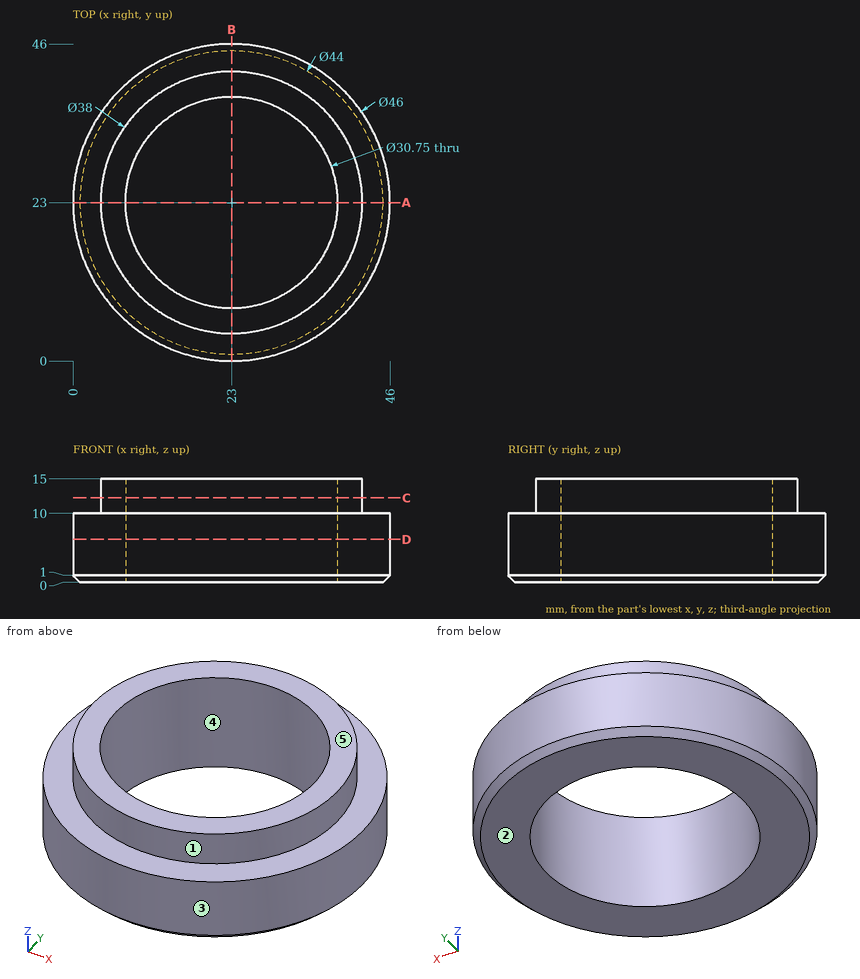
Design review of the part shown in the three views and the two pictorial views. Dimensions are in mm from the part's minimum x, y and z. A direction names the side the tool comes from. Round coordinates to 2 decimals unless told otherwise and drop trailing zeros. Loops run counter-clockwise (first coordinate to the right, second up) from the corner with the lowest first, then second, coordinate; pieces in that order, holes last.
1) Clearance check with flat-ended pins moving along their axes: P1, Ø1.5, axis at y = 34, z = 2.5, coming from the +X side; P2, Ø8, axis at y = 14, z = 11.5, coming from the +X side; P3, Ø4, axis at x = 19.5, z = 2, coming from the -Y side. State where each tip first meets the part, or that it passes through.
Values follow:
P1: stops at x = 43.59
P2: stops at x = 45.38
P3: stops at y = 0.05
2) Consider section C-C on z = 12.25. State the section outline as (x, y) points (3 decimals).
Values follow:
outline: circle Ø38 at (23, 23); hole circle Ø30.75 at (23, 23)
3) Consider section D-D on z = 6.25. State the section outline as (x, y) points (3 decimals), then the cut area to 3 significant figures.
Values follow:
outline: circle Ø46 at (23, 23); hole circle Ø30.75 at (23, 23)
area: 919 mm2
4) Consider section A-A on y = 23. State the section outline as (x, z) points (3 decimals).
Values follow:
outline: (0, 1) - (1, 0) - (7.625, 0) - (7.625, 15) - (4, 15) - (4, 10) - (0, 10) - close; (38.375, 0) - (45, 0) - (46, 1) - (46, 10) - (42, 10) - (42, 15) - (38.375, 15) - close
5) Tool access review of the marked faces 1 and 2: name each direction out of +Z, -Z, +X, -X, +Y, -Y from which nothing blocks a thin tool from reaching the whole face with its end or side.
Values follow:
face 1: +Z
face 2: -Z, +X, -X, +Y, -Y
6) Wall thickness on line 1 along Y through (x, z) = (23, 6.5) (3 decimals); line 2 along Y through (x, z) = (23, 10.75) (3 decimals); line 3 along X through (y, z) = (34.5, 14): over which ranges is each line inside the solid? List them lowest first.
Values follow:
line 1: y = 0 to 7.625, 38.375 to 46
line 2: y = 4 to 7.625, 38.375 to 42
line 3: x = 7.88 to 12.8, 33.2 to 38.12
7) The part is to be moulded in two halves that separate along Y. For the marked faces 3, 4 and 5, say which applies: pulls with the +Y half, pulls with the -Y half, needs draft (parallel to the pull), parting line crosses it, or undercut.
Values follow:
face 3: parting line crosses it
face 4: undercut
face 5: needs draft
